```python
from build123d import *

# Parameters (mm, degrees)
EXTRUDE_387_DEPTH = 7.5
FILLET_1280_R     = 0.6


with BuildPart() as part:
    # 草图1 → Extrude 387 (new body)
    with BuildSketch(Plane(origin=(0, 0, 0), x_dir=(0, 0, -1), z_dir=(1, 0, 0))):
        Polygon((9, 5.196152423), (9, -5.196152423), (0, -10.392304845), (-9, -5.196152423), (-9, 5.196152423), (0, 10.392304845), align=None)
    extrude(amount=EXTRUDE_387_DEPTH)

    # 草图2 → 凸台-旋转1 (revolve)
    with BuildSketch(Plane.XY, mode=Mode.PRIVATE) as revolve_1_sk:
        Polygon((0, 0), (32.5, 0), (32.5, 4.4845), (32.5, 6), (2.5, 6), (0, 6), align=None)
    revolve(revolve_1_sk.sketch.rotate(Axis((0, 0, 0), (1, 0, 0)), 90), axis=Axis((0, 0, 0), (1, 0, 0)))

    # 草图3 → 切除-旋转1 (revolve, cut)
    with BuildSketch(Plane.XY):
        Polygon((0, 9), (3.690598923, 15.392304845), (3.690598923, 20.392304845), (-10, 20.392304845), (-10, 9), align=None)
    revolve(axis=Axis((0, 0, 0), (1, 0, 0)), mode=Mode.SUBTRACT)

    # 草图4 → 切除-旋转3 (revolve, cut)
    with BuildSketch(Plane.XY, mode=Mode.PRIVATE) as cut_revolve_3_sk:
        Polygon((7.5, 8.315), (6.9, 8.661410162), (6.9, 10.392304845), (7.5, 10.392304845), align=None)
    revolve(cut_revolve_3_sk.sketch.rotate(Axis((0, 0, 0), (1, 0, 0)), 90), axis=Axis((0, 0, 0), (1, 0, 0)), mode=Mode.SUBTRACT)

    # Fillet 1280
    fillet_1280_edges = [part.edges().sort_by_distance(p)[0] for p in [
        (7.5, 0, -6),
    ]]
    fillet(fillet_1280_edges, radius=FILLET_1280_R)


solid = part.part
```
Geometry: final body of the model. Coordinates: model frame, mm. A direction names the side the tool comes from. Coordinates: 2 decimals unless noted, no trailing zeros. Order: outer loops, then holes, each group sorted by start corner. A loop starts at its lowest first (then second) coordinate and runs counter-clockwise, first axis right, second up. Notation, with made-up numbers: (-39.75, 66) - (6.25, 66) arc R11 cw to (6.25, 87) - close; hole circle Ø5 at (46.5, 9). An arc over 180 degrees is marked (long way). Return JSON: item names as keys, results as strings. Group by question number.
1. Pin query (flat end, axial travel): pin 1 (2 mm diameter, centred on x = 11, z = 2, fed in from -Y); pin 2 (1.5 mm diameter, centred on x = 8, y = 5, fed in from +Z); pin 3 (2 mm diameter, centred on x = 11.5, z = -0.5, fed in from +Y). Return the tip coordinate at first contact, or that it passes through.
2. Cut plane A-A (x = 21). Output: boundary loops of the cut face in (y, z).
3. Set-up query: faces 1 (the face through (0, 0, 0)), 2 (the face through (6.9, 8.4, 2.7)). Return all of +Z, -Z, +X, -X, +Y, -Y with unobstructed straight access to the full face (end or side cutting, diameter ignored); none if empty.
4. Material intervals for line 1 along X through (y, z) = (6.5, -0.5); line 2 along Z through (x, y) = (27.5, 3); line 3 along X through (y, z) = (-7, -5.5), sorted ascending. Write a range as [from, to].
Resolved:
{
 "1": {"pin 1": "stops at y = -5.92", "pin 2": "stops at z = 7.03", "pin 3": "stops at y = 6"},
 "2": {"outline": "circle Ø12 at (0, 0)"},
 "3": {"face 1": "+Z, -Z, -X, +Y, -Y", "face 2": "+X"},
 "4": {"line 1": "x = [0, 7.51]", "line 2": "z = [-5.2, 5.2]", "line 3": "x = [0, 6.9]"}
}
